Source: CAD feature listing. Evaluate the final solid. Frame: model axes, mm. A direction names the side the tool comes from. Coordinates: 2 decimals unless noted, no trailing zeros. Write each loop counter-clockwise with the first axis right and the second up, starting at its lowest first coordinate (ties: lowest second). Pieces come first, ordered by that corner, then holes. Notation, with made-up numbers: (9.25, -24) - (68.25, -24) arc R29 cw to (68.25, 6) - close; hole circle Ø1 at (15.25, -33). An arc over 180 degrees is marked (long way). One line per item, written item: value.
from build123d import *

# Parameters (mm, degrees)
SKETCH_1_R      = 3.55
SKETCH_3_R      = 4
EXTRUDE_1_DEPTH = 35


with BuildPart() as part:
    # 扫描1: sweep along a path in 草图2
    with BuildLine(Plane(origin=(0, 0, 0), x_dir=(1, 0, 0), z_dir=(0, 1, 0))) as sweep_1_path:
        Line((0, 0), (0, 56.45))
        ThreePointArc((0, 56.45), (43, 99.45), (86, 56.45))
        Line((86, 56.45), (86, 0))
    # 草图1 → 扫描1 (sweep)
    with BuildSketch(Plane.XY):
        Circle(SKETCH_1_R)
    sweep(path=sweep_1_path.line)

    # 草图3 → 凸台-拉伸1 (add)
    with BuildSketch(Plane.XY):
        Circle(SKETCH_3_R)
        with Locations((86, 0)):
            Circle(SKETCH_3_R)
    extrude(amount=-EXTRUDE_1_DEPTH)


solid = part.part
1) Reachability of faces 1 (the cylindrical face through (82.614, -1.066, -45.575)), 2 (the flat face through (86, 0, 0)), 3 (the cylindrical face through (82, 0, -17)) from +Z, -Z, +X, -X, +Y, -Y: full face, straight path, thin tool, end or side. Return the list, or none.
Values found:
face 1: none
face 2: +Z, +X, -X, +Y, -Y
face 3: +Z
2) Section query C-C on z = -6.5. Output: boundary loops of the cut face in (x, y).
Values found:
outline: circle Ø8 at (0, 0); circle Ø8 at (86, 0)
3) Section query A-A on z = -43. Output: boundary loops of the cut face in (x, y), then the cut area to 3 significant figures.
Values found:
outline: circle Ø7.1 at (0, 0); circle Ø7.1 at (86, 0)
area: 79.2 mm2
4) Material intervals for line 1 (X direction, y = 2.25, z = -82); line 2 (X direction, y = 1.75, z = -32.5); line 3 (Z direction, x = 51, y = -0.25), sorted ascending.
Values found:
line 1: 5.05 to 11.89, 74.11 to 80.95
line 2: -3.6 to 3.6, 82.4 to 89.6
line 3: -102.3 to -95.09
5) Draft query along X for faces 4 (the flat face through (0, 0, 0)), 5 (the cylindrical face through (-0.867, -3.905, -17.255)). Return one class per face: released by +X, released by -X, zero draft, split by the parting line, or undercut.
Values found:
face 4: zero draft
face 5: undercut
6) Section query B-B on y = 0. Output: boundary loops of the cut face in (x, z), then the cut area to 3 significant figures.
Values found:
outline: (-4, -35) - (-3.55, -35) - (-3.55, -56.45) arc R46.55 ccw to (89.55, -56.45) - (89.55, -35) - (90, -35) - (90, 0) - (82, 0) - (82, -35) - (82.45, -35) - (82.45, -56.45) arc R39.45 cw to (3.55, -56.45) - (3.55, -35) - (4, -35) - (4, 0) - (-4, 0) - close
area: 1,820 mm2
7) Contact query for flat-ended pins moving along their axis: P1, Ø4, axis at y = 1, z = -50, coming from the +X side; P2, Ø1, axis at y = 2, z = -65, coming from the -X side. Output: stop coordinate, or through.
Values found:
P1: x = 89.55
P2: x = -2.44
